Verification items for this drawing (mm, ordinates from the low corner). A direction names the side the tool comes from. Coordinates: 2 decimals unless noted, no trailing zeros. Order: outer loops, then holes, each group sorted by start corner. A loop starts at its lowest first (then second) coordinate and runs counter-clockwise, first axis right, second up. Notation, with made-up numbers: M -9.5,9 L 35.5,9 A25 ccw 35.5,40 Z; hole C -9,-31.75 d11. An arc over 180 degrees is marked long. One line per item, written item: value. Start each with the question number.
1) Access from +Z, -Z, +X, -X, +Y, -Y to the whole of each face (thin tool, end or side, straight path). Record for the marked faces 5 and 6.
2) Sectioned sample at D-D, the plane y = 80. Enter the section's corners in (x, z).
3) Go/stop test with flat-tipped pins: P1, Ø15.5, axis at x = 42, y = 100, coming from the -Z side; P2, Ø1.5, axis at y = 100, z = 11, coming from the +X side. Record where each tip stops, or that it passes through.
4) Sectioned sample at A-A, the plane x = 52. Enter the section's corners in (y, z), then the cut area to 3 significant figures.
5) Sectioned sample at C-C, the plane x = 42. Enter the section's corners in (y, z).
6) Thickness scan on L1, parallel to Y at x = 42, z = 36; L2, parallel to Z at x = 24, y = 31.5; L3, parallel to X at y = 85, z = 30.5. Record the ranges inside material, lowest first. Write a range as from..to.
7) Draft check along Z on the marked faces 1, 2, 3 and 4. Enter one of: pulls with the +Z half, pulls with the -Z half, needs draft (parallel to the pull), parting line crosses it, or undercut.
8) Sectioned sample at B-B, the plane y = 100. Enter the section's corners in (x, z), then the cut area to 3 significant figures.
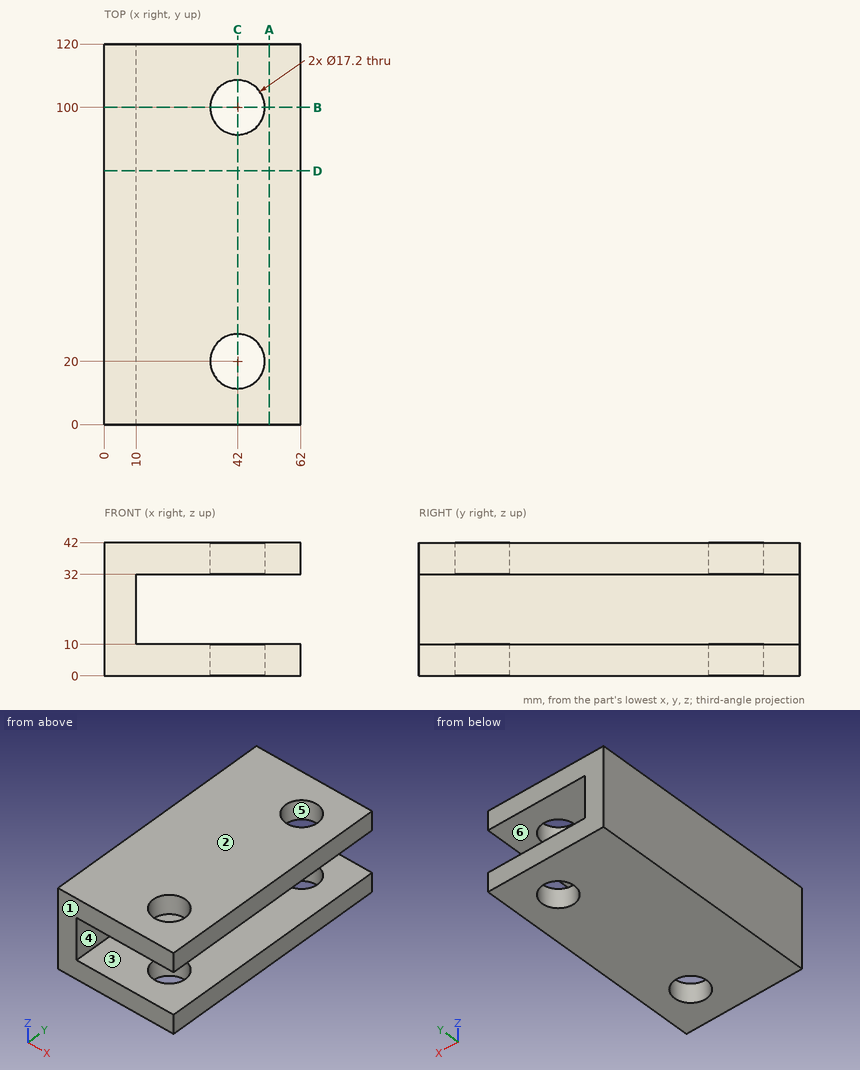
Final values:
1. face 5: +Z, -Z
1. face 6: +X, +Y, -Y
2. outline: M 0,0 L 62,0 L 62,10 L 10,10 L 10,32 L 62,32 L 62,42 L 0,42 Z
3. P1: passes through
3. P2: stops at x = 10
4. outline: M 0,0 L 120,0 L 120,10 L 0,10 Z; M 0,32 L 120,32 L 120,42 L 0,42 Z
4. area: 2,400 mm^2
5. outline: M 0,0 L 11.4,0 L 11.4,10 L 0,10 Z; M 0,32 L 11.4,32 L 11.4,42 L 0,42 Z; M 28.6,0 L 91.4,0 L 91.4,10 L 28.6,10 Z; M 28.6,32 L 91.4,32 L 91.4,42 L 28.6,42 Z; M 108.6,0 L 120,0 L 120,10 L 108.6,10 Z; M 108.6,32 L 120,32 L 120,42 L 108.6,42 Z
6. L1: y = 0..11.4, 28.6..91.4, 108.6..120
6. L2: z = 0..10, 32..42
6. L3: x = 0..10
7. face 1: needs draft
7. face 2: pulls with the +Z half
7. face 3: undercut
7. face 4: undercut
8. outline: M 0,0 L 33.4,0 L 33.4,10 L 10,10 L 10,32 L 33.4,32 L 33.4,42 L 0,42 Z; M 50.6,0 L 62,0 L 62,10 L 50.6,10 Z; M 50.6,32 L 62,32 L 62,42 L 50.6,42 Z
8. area: 1,120 mm^2
